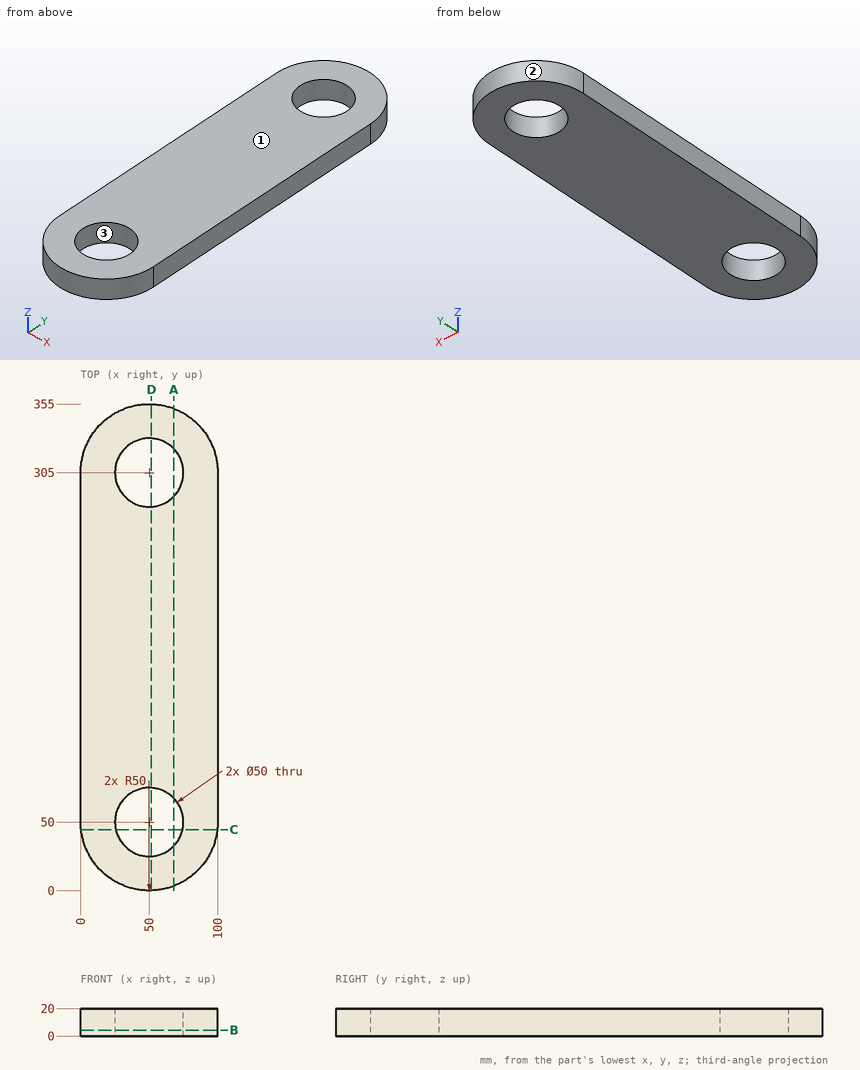
Part print with two shaded views. Sizes in mm from the minimum x, y, z corner. Round coordinates to 2 decimals unless told otherwise and drop trailing zeros. Write each loop counter-clockwise with the first axis right and the second up, starting at its lowest first coordinate (ties: lowest second). Pieces come first, ordered by that corner, then holes. Notation, with made-up numbers: (5, 33) -> (62, 33) arc R28 cw to (62, 55) -> close; hole circle Ø7 at (-12.5, -31.5). An arc over 180 degrees is marked (long way). Use one line per item in the form item = value.
Q1. Band-saw the part on B-B, the plane z = 4.25. Write the cut outline in (x, y), then the cut area to 3 significant figures.
Conclusion:
outline = (0, 50) arc R50 ccw to (100, 50) -> (100, 305) arc R50 ccw to (0, 305) -> close; hole circle Ø50 at (50, 50); hole circle Ø50 at (50, 305)
area = 29,400 mm²
Q2. Drill centre lines: L1, parallel to Y at x = 50, z = 6.75; L2, parallel to Y at x = 68, z = 12.25; L3, parallel to X at y = 33.5, z = 13. Where is each one in solid material? Low to high.
Conclusion:
L1 = 0 to 25, 75 to 280, 330 to 355
L2 = 3.35 to 32.65, 67.35 to 287.65, 322.35 to 351.65
L3 = 2.8 to 31.22, 68.78 to 97.2
Q3. Band-saw the part on A-A, the plane x = 68. Write the cut outline in (y, z), then the cut area to 3 significant figures.
Conclusion:
outline = (3.35, 0) -> (32.65, 0) -> (32.65, 20) -> (3.35, 20) -> close; (67.35, 0) -> (287.65, 0) -> (287.65, 20) -> (67.35, 20) -> close; (322.35, 0) -> (351.65, 0) -> (351.65, 20) -> (322.35, 20) -> close
area = 5,580 mm²
Q4. Two-plate mould, pull along X, no slides. Class the marked faces 1, 2 and 3: released by +X, released by -X, zero draft, split by the parting line, or undercut.
Conclusion:
face_1 = zero draft
face_2 = split by the parting line
face_3 = undercut
Q5. Band-saw the part on D-D, the plane x = 51.5. Write the cut outline in (y, z), then the cut area to 3 significant figures.
Conclusion:
outline = (0.02, 0) -> (25.05, 0) -> (25.05, 20) -> (0.02, 20) -> close; (74.95, 0) -> (280.05, 0) -> (280.05, 20) -> (74.95, 20) -> close; (329.95, 0) -> (354.98, 0) -> (354.98, 20) -> (329.95, 20) -> close
area = 5,100 mm²
Q6. Drop flat-ended pins along their axis: P1, Ø6, axis at x = 21, z = 10.5, coming from the +Y side; P2, Ø2, axis at x = 72, y = 311, coming from the +Z side; P3, Ø10, axis at x = 83.5, z = 2, coming from the -Y side; P4, Ø1, axis at x = 88, y = 196, coming from the -Z side. Give the stop position or say it passes through.
Conclusion:
P1 = 347.71
P2 = through
P3 = 8.92
P4 = 0
Q7. Band-saw the part on C-C, the plane y = 44.5. Write the cut outline in (x, z).
Conclusion:
outline = (0.3, 0) -> (25.61, 0) -> (25.61, 20) -> (0.3, 20) -> close; (74.39, 0) -> (99.7, 0) -> (99.7, 20) -> (74.39, 20) -> close
